from build123d import *

# Parameters (mm, degrees)
SKETCH1_R           = 90
SKETCH1_R_2         = 50
BOSS_EXTRUDE1_DEPTH = 60
CHAMFER1_SIZE       = 2


with BuildPart() as part:
    # Sketch1 → Boss-Extrude1 (new body)
    with BuildSketch(Plane.XY):
        Circle(SKETCH1_R)
        Circle(SKETCH1_R_2, mode=Mode.SUBTRACT)
    extrude(amount=BOSS_EXTRUDE1_DEPTH)

    # Chamfer1
    chamfer1_edges = [part.edges().sort_by_distance(p)[0] for p in [
        (-90, 0, 0),
        (-90, 0, 60),
        (-50, 0, 0),
        (-50, 0, 60),
    ]]
    chamfer(chamfer1_edges, length=CHAMFER1_SIZE)


solid = part.part
Could you check a few things on this model? Use its own coordinates, in mm. Give positions to 0.01 mm unless a question says otherwise; leave off trailing zeros. Order: outer loops, then holes, each group sorted by start corner. A loop starts at its lowest first (then second) coordinate and runs counter-clockwise, first axis right, second up. Notation, with made-up numbers: (43, 46) - (62, 46) arc R19 ccw to (62, 61) - close; hole circle Ø8 at (-7, 62.5). An arc over 180 degrees is marked (long way). Return JSON: item names as keys, results as strings. Group by question number.
Q1. Please list where these lines run through material, in increasing order: line 1 along X through (y, z) = (-1.5, 17); line 2 along Y through (x, z) = (0, 31.5); line 3 along Y through (x, z) = (19, 13.5). Write a range as [from, to].
Q2. Thinking about a two-plate mould opening in Y: for faces 1 (the face through (-10.866, -48.933, 1.875)), 2 (the face through (38, -38, 0)), 3 (the face through (41.53, -79.845, 29.608)), which applies, pulls with the +Y half, pulls with the -Y half, needs draft (parallel to the pull), parting line crosses it, or undercut?
Q3. Suppose I cut it at C-C, the plane z = 50. Please give me the cut outline in (x, y), and give its area (3 significant figures).
Q4. Will these pins go through, and if not, where does the flat tip stop? pin 1 Ø4 at (y, z) = (-70.5, 31.5) entering from +X; pin 2 Ø1 at (x, z) = (-67.5, 14.5) entering from -Y; pin 3 Ø1.5 at (x, z) = (55, 52.5) entering from -Y.
Q5. Suppose I cut it at A-A, the plane y = 0. Please give me the cut outline in (x, z).
Resolved:
{
 "1": {"line 1": "x = [-89.99, -49.98], [49.98, 89.99]", "line 2": "y = [-90, -50], [50, 90]", "line 3": "y = [-87.97, -46.25], [46.25, 87.97]"},
 "2": {"face 1": "undercut", "face 2": "needs draft", "face 3": "parting line crosses it"},
 "3": {"outline": "circle Ø180 at (0, 0); hole circle Ø100 at (0, 0)", "area": "17,600 mm2"},
 "4": {"pin 1": "stops at x = 58.38", "pin 2": "stops at y = -60.09", "pin 3": "stops at y = -71.81"},
 "5": {"outline": "(-90, 2) - (-88, 0) - (-52, 0) - (-50, 2) - (-50, 58) - (-52, 60) - (-88, 60) - (-90, 58) - close; (50, 2) - (52, 0) - (88, 0) - (90, 2) - (90, 58) - (88, 60) - (52, 60) - (50, 58) - close"}
}
